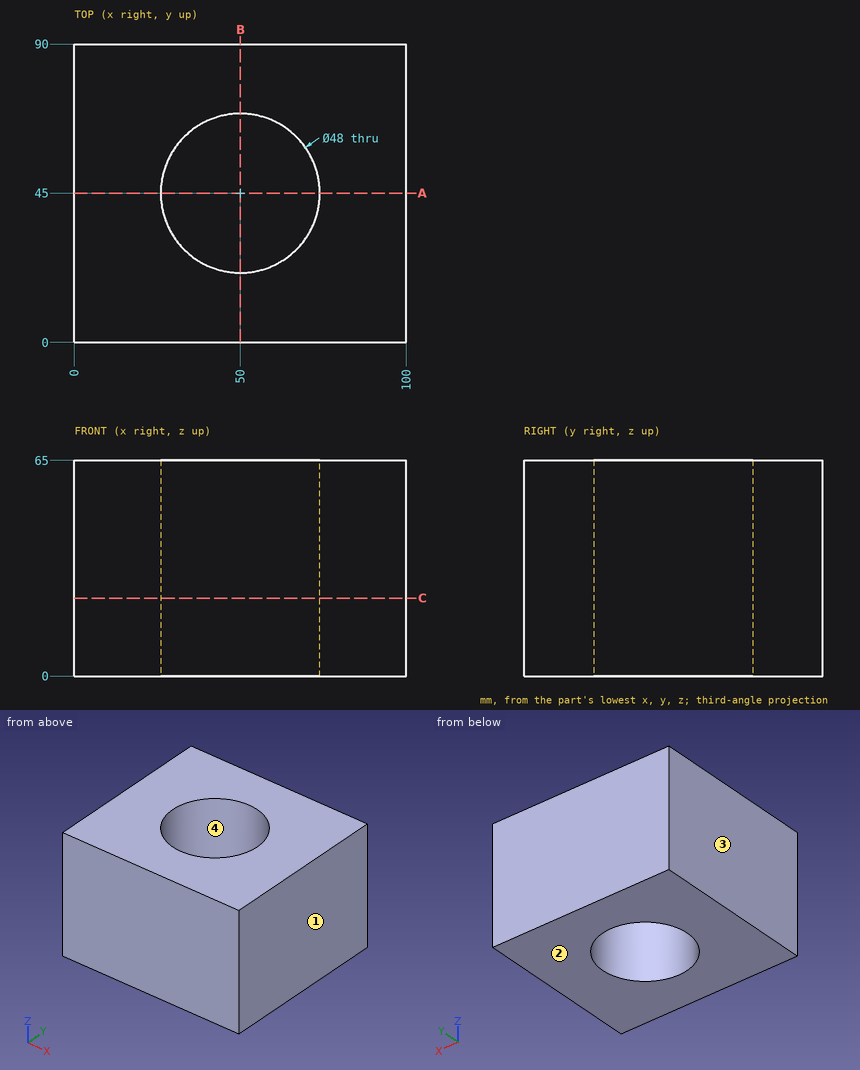
Drawing for the job (mm, zero at the part's lowest x, y, z). Round coordinates to 2 decimals unless told otherwise and drop trailing zeros. Write each loop counter-clockwise with the first axis right and the second up, starting at its lowest first coordinate (ties: lowest second). Pieces come first, ordered by that corner, then holes. Notation, with made-up numbers: (-9, 1) - (42, 1) arc R16 cw to (42, 22) - close; hole circle Ø6 at (59.25, 72). An arc over 180 degrees is marked (long way). Write item = value, one per line. Start each with the question number.
Q1. Drop a flat-ended pin along its axis: pin 1 (4 mm diameter, centred on y = 14, z = 7.5, fed in from -X). Give the stop position or say it passes through.
Q2. Band-saw the part on C-C (z = 23.5). Give the cut face in (x, y), then the cut area to 3 significant figures.
Q3. Band-saw the part on B-B (x = 50). Give the cut face in (y, z).
Q4. Mould opens along X. For the marked faces 1, 2, 3 and 4 say: pulls with the +X half, pulls with the -X half, needs draft (parallel to the pull), parting line crosses it, or undercut.
Q5. Probe L1, parallel to Y at x = 50, z = 44; L2, parallel to Y at x = 66.5, z = 49; L3, parallel to X at y = 36, z = 11. List the from-to ranges inside material, lowest first. Write a range as from..to.
Q6. Band-saw the part on A-A (y = 45). Give the cut face in (x, z).
Answers below:
q1.pin_1 = 0
q2.outline = (0, 0) - (100, 0) - (100, 90) - (0, 90) - close; hole circle Ø48 at (50, 45)
q2.area = 7,190 mm2
q3.outline = (0, 0) - (21, 0) - (21, 65) - (0, 65) - close; (69, 0) - (90, 0) - (90, 65) - (69, 65) - close
q4.face_1 = pulls with the +X half
q4.face_2 = needs draft
q4.face_3 = pulls with the -X half
q4.face_4 = undercut
q5.L1 = 0..21, 69..90
q5.L2 = 0..27.57, 62.43..90
q5.L3 = 0..27.75, 72.25..100
q6.outline = (0, 0) - (26, 0) - (26, 65) - (0, 65) - close; (74, 0) - (100, 0) - (100, 65) - (74, 65) - close
